Input: part model. Units: mm. Frame: model coordinates. Face numbers are marked on the shaded views. Give positions to 0.01 mm unless a question says otherwise; leave off trailing zeros. Loops run counter-clockwise (first coordinate to the right, second up) from the corner with the lowest first, then second, coordinate; pieces in that order, holes last. Notation, with made-up numbers: M -13.5,15 L -2.5,15 A29 cw -2.5,35 Z; hole C 55,-7.5 d9. An arc over 180 degrees is marked long. Answer as a JSON object with one key per item and string values. Group by question number.
1) Section query B-B on x = -7. Return loops of the section in (y, z).
2) Section query C-C on z = -35.5. Return loops of the section in (x, y).
3) Section query D-D on x = -22.5. Return loops of the section in (y, z), plus the area to 3 significant figures.
4) Ray query, L1, parallel to Y at x = 0, z = 1.5; L2, parallel to Y at x = 0, z = -12; L3, parallel to X at y = 13.5, z = 6.5. Return the intervals inside material, ascending.
5) Section query A-A on y = 0. Return loops of the section in (x, z), plus the area to 3 significant figures.
6) First-contact query: P1, Ø12, axis at y = -8.5, z = 12, coming from the -X side; P2, Ø4, axis at x = -10, z = -36.5, coming from the +Y side; P3, Ø12, axis at x = 20.5, z = -12.5, coming from the -Y side. Flat tips, straight axial feed; report the tip coordinate or a pass-through.
7) Draft query along Y for the marked faces 1, 2 and 3. Return one class per face: +Y half, -Y half, draft (parallel to the pull), parting line (faces both ways), or undercut.
from build123d import *

# Parameters (mm, degrees)
SKETCH1_R             = 30
SKETCH1_R_2           = 21.5
BOSS_EXTRUDE1_DEPTH   = 50
M6_TAPPED_HOLE1_D     = 5
M6_TAPPED_HOLE1_DEPTH = 18
M6_TAPPED_HOLE1_TIP   = 1.502151548
BOSS_EXTRUDE2_START   = 24
SKETCH4_R             = 25
SKETCH4_R_2           = 21.5
BOSS_EXTRUDE2_DEPTH   = 24


with BuildPart() as part:
    # Sketch1 → Boss-Extrude1 (new body)
    with BuildSketch(Plane.XY):
        Circle(SKETCH1_R)
        Circle(SKETCH1_R_2, mode=Mode.SUBTRACT)
    extrude(amount=-BOSS_EXTRUDE1_DEPTH)

    # M6 Tapped Hole1
    with Locations(Plane(origin=(3.471069712, 29.798518001, -40), x_dir=(0.993283933364, -0.115702323745, 0), z_dir=(0.115702323745, 0.993283933364, 0))):
        with Locations((0, 0)):
            Hole(M6_TAPPED_HOLE1_D / 2, depth=M6_TAPPED_HOLE1_DEPTH)
            with Locations((0, 0, -(M6_TAPPED_HOLE1_DEPTH + M6_TAPPED_HOLE1_TIP / 2))):  # 118° drill point
                Cone(0, M6_TAPPED_HOLE1_D / 2, M6_TAPPED_HOLE1_TIP, mode=Mode.SUBTRACT)

    # Sketch4 → Boss-Extrude2 (add)
    with BuildSketch(Plane.XY.offset(BOSS_EXTRUDE2_START)):
        Circle(SKETCH4_R)
        Circle(SKETCH4_R_2, mode=Mode.SUBTRACT)
    extrude(amount=-BOSS_EXTRUDE2_DEPTH)


solid = part.part
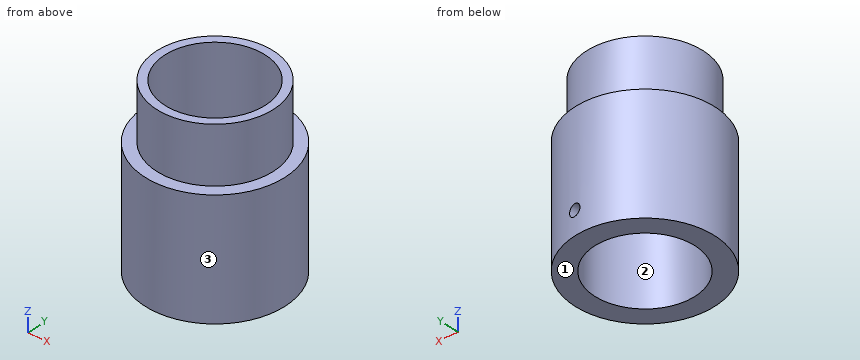
Output:
{
 "1": {"outline": "M -29.17,-50 L -20.33,-50 L -20.33,24 L -24,24 L -24,0 L -29.17,0 Z; M 20.33,-50 L 29.17,-50 L 29.17,0 L 24,0 L 24,24 L 20.33,24 Z"},
 "2": {"outline": "C 0,0 d60; hole C 0,0 d43"},
 "3": {"outline": "M -19.84,-50 L 19.84,-50 L 19.84,0 L 10.9,0 L 10.9,24 L -10.9,24 L -10.9,0 L -19.84,0 Z", "area": "2,510 mm^2"},
 "4": {"L1": "y = -25 to -21.5, 21.5 to 25", "L2": "y = -30 to -21.5, 21.5 to 30", "L3": "x = -21.04 to -16.73, 16.73 to 21.04"},
 "5": {"outline": "M -30,-50 L -21.5,-50 L -21.5,24 L -25,24 L -25,0 L -30,0 Z; M 21.5,-50 L 30,-50 L 30,0 L 25,0 L 25,24 L 21.5,24 Z", "area": "1,020 mm^2"},
 "6": {"P1": "stops at x = -24.87", "P2": "stops at y = 28.91", "P3": "stops at y = -26.26"},
 "7": {"face 1": "draft", "face 2": "undercut", "face 3": "parting line"}
}
